Design review of the part built by this model. Coordinates are the model's own, in mm. Coordinates: 2 decimals unless noted, no trailing zeros. Order: outer loops, then holes, each group sorted by start corner. A loop starts at its lowest first (then second) coordinate and runs counter-clockwise, first axis right, second up. Notation, with made-up numbers: M -5.5,-38 L 1.5,-38 A22 cw 1.5,-26 Z; hole C 34,86 d6. An arc over 180 degrees is marked long. Answer in a Markdown table with one row per item.
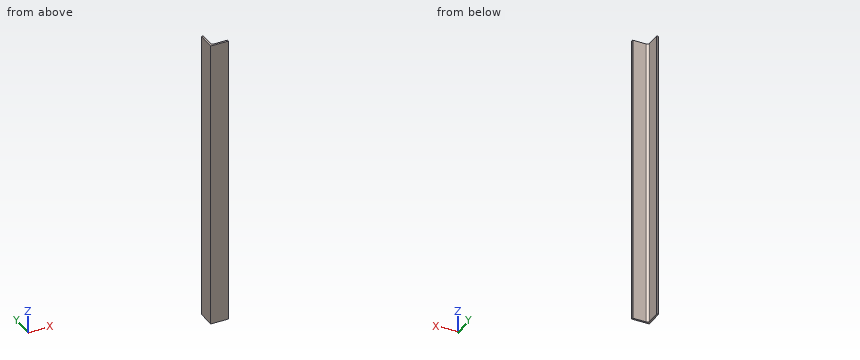
from build123d import *

# Parameters (mm, degrees)
BOSS_EXTRUDE1_DEPTH = 660


with BuildPart() as part:
    # Sketch1 → Boss-Extrude1 (new body)
    with BuildSketch(Plane.XY):
        with BuildLine():
            Line((0, 0), (0, 40))
            Line((0, 40), (2.666666667, 40))
            ThreePointArc((2.666666667, 40), (3.609475708, 39.609475708), (4, 38.666666667))
            Line((4, 38.666666667), (4, 9))
            ThreePointArc((4, 9), (5.464466094, 5.464466094), (9, 4))
            Line((9, 4), (38.666666667, 4))
            ThreePointArc((38.666666667, 4), (39.609475708, 3.609475708), (40, 2.666666667))
            Line((40, 2.666666667), (40, 0))
            Line((40, 0), (0, 0))
        make_face()
    extrude(amount=BOSS_EXTRUDE1_DEPTH)


solid = part.part
(1) Add section A-A, the plane z = 315. Give the boundary of the cut face in (x, y), and give its area (3 significant figures).
Return value:
| item | result |
|---|---|
| outline | M 0,0 L 40,0 L 40,2.67 A1.33 ccw 38.67,4 L 9,4 A5 cw 4,9 L 4,38.67 A1.33 ccw 2.67,40 L 0,40 Z |
| area | 309 mm2 |
(2) Add section B-B, the plane y = 28. Give the boundary of the cut face in (x, z), and give its area (3 significant figures).
Return value:
| item | result |
|---|---|
| outline | M 0,0 L 4,0 L 4,660 L 0,660 Z |
| area | 2,640 mm2 |
(3) For line 1 along X through (y, z) = (28.5, 35); line 2 along X through (y, z) = (6, 517), list the stretches that pass through material, from the lowest coordinate up. Write a range as from..to.
Return value:
| item | result |
|---|---|
| line 1 | x = 0..4 |
| line 2 | x = 0..5 |
(4) Insertion check: pin 1 Ø1.5 at (x, z) = (26, 323.5) entering from +Y; pin 2 Ø6 at (x, y) = (6, 21) entering from -Z; pin 3 Ø15 at (y, z) = (27.5, 349) entering from +X; pin 4 Ø2 at (x, z) = (8.5, 504) entering from +Y. Each pin has a flat end and moves straight along its axis. Give the tip position at first contact, or say it passes through.
Return value:
| item | result |
|---|---|
| pin 1 | stops at y = 4 |
| pin 2 | stops at z = 0 |
| pin 3 | stops at x = 4 |
| pin 4 | stops at y = 4.23 |
